Source: CAD feature listing. Evaluate the final solid. Frame: model axes, mm. Face numbers are marked on the shaded views. Round coordinates to 2 decimals unless told otherwise and drop trailing zeros. Write each loop counter-clockwise with the first axis right and the second up, starting at its lowest first coordinate (ties: lowest second). Pieces come first, ordered by that corner, then holes. Notation, with made-up numbers: (81, -39) -> (108, -39) arc R17 ccw to (108, -16) -> close; hole circle Ø9 at (57, -39.5). An arc over 180 degrees is marked (long way). Return JSON: item names as keys, results as strings. Group by question number.
from build123d import *

# Parameters (mm, degrees)
SKETCH1_R               = 9
BOSS_EXTRUDE1_DEPTH     = 44
CUT_EXTRUDE1_DEPTH      = 46.803929962
LPATTERN1_COUNT         = 8
LPATTERN1_PITCH         = 8
CUT_EXTRUDE2_DEPTH      = 46.803929962
CUT_EXTRUDE2_DEPTH_BACK = 46.803929962
SKETCH4_W               = 11.104020724
SKETCH4_H               = 55.76293723


with BuildPart() as part:
    # Sketch1 → Boss-Extrude1 (new, symmetric)
    with BuildSketch(Plane.XY):
        Circle(SKETCH1_R)
    extrude(amount=BOSS_EXTRUDE1_DEPTH, both=True)

    # Sketch2 → Cut-Extrude1 (cut, symmetric)
    with BuildSketch(Plane(origin=(0, 0, 0), x_dir=(1, 0, 0), z_dir=(0, 1, 0))):
        Polygon((9, -34), (1.125, -31.133734405), (1.125, -30.143622784), (9, -27.277357189), align=None)
    cut_extrude1 = extrude(amount=CUT_EXTRUDE1_DEPTH, both=True, mode=Mode.SUBTRACT)

    # LPattern1: Cut-Extrude1 ×8
    with Locations(*[(0, 0, -i * LPATTERN1_PITCH) for i in range(1, LPATTERN1_COUNT)]):
        add(cut_extrude1, mode=Mode.SUBTRACT)

    # Sketch4 → Cut-Extrude2 (cut, two sides: drawn at the far end of the back side and taken through both)
    with BuildSketch(Plane(origin=(0, 0, 0), x_dir=(1, 0, 0), z_dir=(0, 1, 0)).offset(-CUT_EXTRUDE2_DEPTH_BACK)):
        with Locations((11.693935952, -1.197060718)):
            Rectangle(SKETCH4_W, SKETCH4_H)
    extrude(amount=CUT_EXTRUDE2_DEPTH + CUT_EXTRUDE2_DEPTH_BACK, mode=Mode.SUBTRACT)


solid = part.part
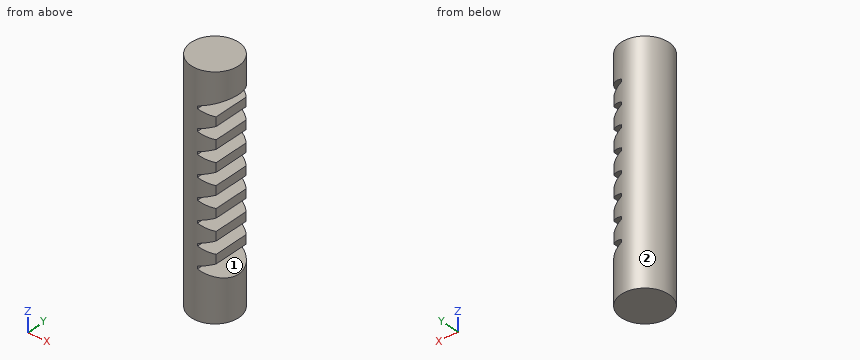
Item 1: Material intervals for probe 1 along X at (y, z) = (-1.25, 3); probe 2 along Y at (x, z) = (1, 15); probe 3 along Y at (x, z) = (7.25, -39.5), sorted ascending.
Item 2: Pull-direction query (Y, two-part tool) for the marked faces 1 and 2; classes: +Y half, -Y half, draft (parallel to the pull), parting line (faces both ways), or undercut.
Item 3: Cut plane B-B on x = 2. Give the number of separate pieces and of enclosed holes in the cut face, and give its area (3 significant figures).
Item 4: Cut plane A-A on z = 37.5. Output: boundary loops of the cut face in (x, y), and give its area (3 significant figures).
Item 5: First-contact query: pin 1 Ø10 at (y, z) = (-1, 11) entering from +X; pin 2 Ø4 at (x, z) = (-6, -4.5) entering from +Y; pin 3 Ø10 at (x, z) = (-6, -31.5) entering from +Y. Flat tips, straight axial feed; report the tip coordinate or a pass-through.
Item 6: Cut plane C-C on z = -4.5. Output: boundary loops of the cut face in (x, y).
Here are the results:
{
 "1": {"probe 1": "x = -8.91 to 6.14", "probe 2": "y = -8.94 to 8.94", "probe 3": "y = -5.33 to 5.33"},
 "2": {"face 1": "draft", "face 2": "parting line"},
 "3": {"separate pieces": "9", "enclosed holes": "0", "area": "1,320 mm^2"},
 "4": {"outline": "circle Ø18 at (0, 0)", "area": "254 mm^2"},
 "5": {"pin 1": "stops at x = 6.14", "pin 2": "stops at y = 8.06", "pin 3": "stops at y = 8.94"},
 "6": {"outline": "(6.14, -6.58) -> (6.14, 6.58) arc R9 ccw (long way) to start"}
}
